```python
from build123d import *

# Parameters (mm, degrees)
SKETCH_1_W      = 80
SKETCH_1_H      = 80
EXTRUDE_1_DEPTH = 30
SKETCH_2_R      = 31.5
EXTRUDE_2_DEPTH = 10


with BuildPart() as part:
    # 草图1 → 凸台-拉伸1 (new body)
    with BuildSketch(Plane.XY):
        Rectangle(SKETCH_1_W, SKETCH_1_H)
    extrude(amount=EXTRUDE_1_DEPTH)

    # 草图2 → 凸台-拉伸2 (add)
    with BuildSketch(Plane.XY.offset(30)):
        Circle(SKETCH_2_R)
    extrude(amount=EXTRUDE_2_DEPTH)


solid = part.part
```
CAD build for the part. Positions are in the model's coordinates, mm. A direction names the side the tool comes from. Give positions to 0.01 mm unless a question says otherwise; leave off trailing zeros. Order: outer loops, then holes, each group sorted by start corner. A loop starts at its lowest first (then second) coordinate and runs counter-clockwise, first axis right, second up.
(1) Flat gauge pins, fed straight in: pin 1 (8 mm diameter, centred on y = -23, z = 35.5, fed in from +X); pin 2 (2 mm diameter, centred on x = -30, y = 26, fed in from +Z); pin 3 (1.5 mm diameter, centred on x = -19, z = 34, fed in from -Y). Where does each tip first touch, or does it go through?
(2) Tool access for faces 1 (the flat face through (-1, 1, 0)), 2 (the flat face through (-18, 27, 30)): list every direction of +Z, -Z, +X, -X, +Y, -Y with a clear straight run to the whole face (end or side of a thin tool).
(3) Drill centre lines: L1, parallel to X at y = 1, z = 36; L2, parallel to Z at x = 36, y = -14; L3, parallel to Y at x = 29, z = 31. Where is each one in solid material? Low to high.
(4) Saw through at A-A, the plane y = 0. Give the cut face in (x, z).
(5) Mould opens along Y. For faces 3 (the cylindrical face through (-4.101, 31.232, 34.93)), 4 (the flat face through (-1, 40, 15)), 5 (the flat face through (0, 0, 40)) say: released by +Y, released by -Y, zero draft, split by the parting line, or undercut.
(6) Saw through at C-C, the plane z = 34. Give the cut face in (x, y).
Results found:
1. pin 1: stops at x = 25.12
1. pin 2: stops at z = 30
1. pin 3: stops at y = -25.67
2. face 1: -Z, +X, -X, +Y, -Y
2. face 2: +Z
3. L1: x = -31.48 to 31.48
3. L2: z = 0 to 30
3. L3: y = -12.3 to 12.3
4. outline: (-40, 0) - (40, 0) - (40, 30) - (31.5, 30) - (31.5, 40) - (-31.5, 40) - (-31.5, 30) - (-40, 30) - close
5. face 3: split by the parting line
5. face 4: released by +Y
5. face 5: zero draft
6. outline: circle Ø63 at (0, 0)
